from build123d import *

# Parameters (mm, degrees)
BOSS_EXTRUDE1_DEPTH = 6


with BuildPart() as part:
    # Sketch1 → Boss-Extrude1 (new body)
    with BuildSketch(Plane.XY):
        with BuildLine():
            Line((0, 0), (15, 0))
            Line((15, 0), (81, 55))
            Line((81, 55), (81, 85))
            Line((81, 85), (66, 100))
            Line((66, 100), (35, 100))
            Line((35, 100), (19, 85))
            ThreePointArc((19, 85), (11.791612432, 41.987757221), (0, 0))
        make_face()
    extrude(amount=BOSS_EXTRUDE1_DEPTH)


solid = part.part
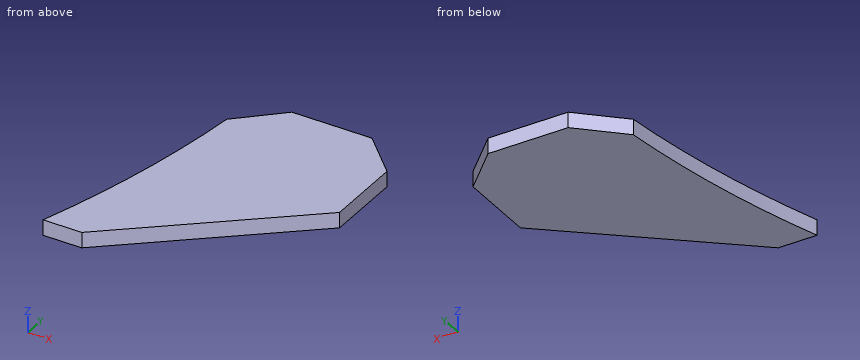
Design review of the part built by this model. Coordinates are the model's own, in mm. Coordinates: 2 decimals unless noted, no trailing zeros. Loops run counter-clockwise (first coordinate to the right, second up) from the corner with the lowest first, then second, coordinate; pieces in that order, holes last. Notation, with made-up numbers: M 32,19.5 L 90,19.5 A15 cw 90,47.5 Z; hole C 66.25,22 d11. An arc over 180 degrees is marked long. Use one line per item in the form item = value.
(1) Consider section C-C (y = 26.5). Write out the cut boundary in (x, z), and give its area (3 significant figures).
Return value:
outline = M 8.01,0 L 46.8,0 L 46.8,6 L 8.01,6 Z
area = 233 mm2
(2) For line 1 along Y through (x, z) = (46, 3.15); line 2 along X through (y, z) = (48, 3.55); line 3 along Y through (x, z) = (52, 4.9), list the stretches that pass through material, from the lowest coordinate up. Write a range as from..to.
Return value:
line_1 = 25.83..100
line_2 = 13.09..72.6
line_3 = 30.83..100
(3) Clearance check with flat-ended pins moving along their axes: P1, Ø1, axis at y = 19.5, z = 3.5, coming from the +X side; P2, Ø3, axis at y = 40.5, z = 3.5, coming from the +X side; P3, Ø3, axis at x = 68.5, z = 1.5, coming from the +Y side. State where each tip first meets the part, or that it passes through.
Return value:
P1 = 39
P2 = 65.4
P3 = 99
(4) Consider section B-B (x = 51). Write out the cut boundary in (y, z), and give its area (3 significant figures).
Return value:
outline = M 30,0 L 100,0 L 100,6 L 30,6 Z
area = 420 mm2
(5) Consider section A-A (z = 4.7). Write out the cut boundary in (x, y), and give its area (3 significant figures).
Return value:
outline = M 0,0 L 15,0 L 81,55 L 81,85 L 66,100 L 35,100 L 19,85 A405 cw Z
area = 4,820 mm2
